from build123d import *

# Parameters (mm, degrees)
BACK_PLATE_DEPTH        = 10
BASE_PLATE_DEPTH        = 10
HOUSING_BOSS_DEPTH      = 50
MOUNTING_HOLES_REACH    = 124.984
MOUNTING_HOLES_SKETCH_R = 7.5
HOUSING_SLOT_PROFILE_W  = 28.353660078
HOUSING_SLOT_PROFILE_H  = 63.245553204
HOUSING_SLOT_CUT_DEPTH  = 20


with BuildPart() as part:
    # Back Plate Profile → Back Plate (new body)
    with BuildSketch(Plane(origin=(0, 0, 0), x_dir=(0, 0, -1), z_dir=(1, 0, 0))):
        with BuildLine():
            Line((-50, -70), (50, -70))
            Line((50, -70), (50, -60))
            Line((50, -60), (34.077790239, 7.981491866))
            ThreePointArc((34.077790239, 7.981491866), (0, 35), (-34.077790239, 7.981491866))
            Line((-34.077790239, 7.981491866), (-50, -60))
            Line((-50, -60), (-50, -70))
        make_face()
    extrude(amount=BACK_PLATE_DEPTH)

    # Base Plate Profile → Base Plate (add)
    with BuildSketch(Plane.XZ.offset(70)):
        Polygon((10, 50), (50, 50), (60, 40), (60, -40), (50, -50), (10, -50), align=None)
    extrude(amount=-BASE_PLATE_DEPTH)

    # Housing Boss Profile → Housing Boss (add)
    with BuildSketch(Plane(origin=(10, 0, 0), x_dir=(0, 0, -1), z_dir=(1, 0, 0))):
        with BuildLine():
            Line((-5, -34.641016151), (-5, -60))
            Line((-5, -60), (5, -60))
            Line((5, -60), (5, -34.641016151))
            ThreePointArc((5, -34.641016151), (0, 35), (-5, -34.641016151))
        make_face()
    extrude(amount=HOUSING_BOSS_DEPTH)

    # Mounting Holes Sketch → Mounting Holes (cut, up to next)
    with BuildSketch(Plane(origin=(0, -60, 0), x_dir=(1, 0, 0), z_dir=(0, 1, 0)), mode=Mode.PRIVATE) as mounting_holes_sk1:
        with Locations(Location((40, 35, 0), (0, 0, 270))):
            Circle(MOUNTING_HOLES_SKETCH_R)
    mounting_holes_tool1 = extrude(mounting_holes_sk1.sketch, amount=-MOUNTING_HOLES_REACH, mode=Mode.PRIVATE) & part.part
    # Mounting Holes Sketch → Mounting Holes (cut, up to next)
    with BuildSketch(Plane(origin=(0, -60, 0), x_dir=(1, 0, 0), z_dir=(0, 1, 0)), mode=Mode.PRIVATE) as mounting_holes_sk2:
        with Locations(Location((40, -35, 0), (0, 0, 270))):
            Circle(MOUNTING_HOLES_SKETCH_R)
    mounting_holes_tool2 = extrude(mounting_holes_sk2.sketch, amount=-MOUNTING_HOLES_REACH, mode=Mode.PRIVATE) & part.part
    add(mounting_holes_tool1.solids().sort_by_distance((40, -60, -35))[0], mode=Mode.SUBTRACT)
    add(mounting_holes_tool2.solids().sort_by_distance((40, -60, 35))[0], mode=Mode.SUBTRACT)

    # Gland Bore Profile → Gland Bore (revolve, cut)
    with BuildSketch(Plane.XY, mode=Mode.PRIVATE) as gland_bore_sk:
        Polygon((0, 0), (60, 0), (60, 25), (50, 25), (50, 20), (40, 20), (0, 20), align=None)
    revolve(gland_bore_sk.sketch.rotate(Axis((0, 0, 0), (1, 0, 0)), 90), axis=Axis((0, 0, 0), (1, 0, 0)), mode=Mode.SUBTRACT)

    # Housing Slot Profile → Housing Slot Cut (cut)
    with BuildSketch(Plane(origin=(60, 0, 0), x_dir=(0, 0, -1), z_dir=(1, 0, 0))):
        with Locations((-29.176830039, 0)):
            Rectangle(HOUSING_SLOT_PROFILE_W, HOUSING_SLOT_PROFILE_H)
        with Locations((29.176830039, 0)):
            Rectangle(HOUSING_SLOT_PROFILE_W, HOUSING_SLOT_PROFILE_H)
    extrude(amount=-HOUSING_SLOT_CUT_DEPTH, mode=Mode.SUBTRACT)


solid = part.part
Model file for the job. Use its own axes, mm. A direction names the side the tool comes from. Give positions to 0.01 mm unless a question says otherwise; leave off trailing zeros. Write each loop counter-clockwise with the first axis right and the second up, starting at its lowest first coordinate (ties: lowest second). Pieces come first, ordered by that corner, then holes. Notation, with made-up numbers: M -11.75,68.5 L 3.25,68.5 A24 cw 3.25,92.5 Z; hole C 35,45 d7. An arc over 180 degrees is marked long. One line per item, written item: value. Start each with the question number.
Q1. Probe probe 1 along Y at (x, z) = (33.5, -15); probe 2 along X at (y, z) = (-65.25, 35); probe 3 along Y at (x, z) = (47.5, -39.5). List the from-to ranges inside material, lowest first. Write a range as [from, to].
Q2. 3-axis set-ups, long thin cutter, end or side, ignore diameter. For faces 1 (the flat face through (10, -41, -27)), 2 (the flat face through (10, -41, 28)), 3 (the flat face through (40, 0, -25)): which of +Z, -Z, +X, -X, +Y, -Y reach the whole face in a straight line?
Q3. Saw through at B-B, the plane y = 11. Write the cut outline in (x, z).
Q4. Drop flat-ended pins along their axis: pin 1 Ø22 at (y, z) = (-11, 23.5) entering from +X; pin 2 Ø2 at (x, y) = (19, 3) entering from -Z; pin 3 Ø13.5 at (x, z) = (37.5, 31) entering from +Y. Give the stop position or say it passes through.
Q5. Saw through at A-A, the plane z = 0. Write the cut outline in (x, y), plus the area to 3 significant figures.
Q6. Saw through at C-C, the plane y = 0. Write the cut outline in (x, z).
Q7. Two-plate mould, pull along Y, no slides. Class faces 4 (the flat face through (50, 20.3, -0.2)), 5 (the flat face through (4.93, -26.49, -42.15)), 6 (the flat face through (55, -65, 45)): +Y half, -Y half, draft (parallel to the pull), parting line (faces both ways), or undercut.
Output values:
1. probe 1: y = [-70, -60], [-31.62, -13.23], [13.23, 31.62]
1. probe 2: x = [0, 32.5], [47.5, 60]
1. probe 3: y = [-70, -60]
2. face 1: -Z, +X
2. face 2: +Z, +X
2. face 3: -Z, +X, +Y
3. outline: M 0,-33.23 L 40,-33.23 L 40,-16.7 L 0,-16.7 Z; M 0,16.7 L 40,16.7 L 40,33.23 L 0,33.23 Z
4. pin 1: stops at x = 50
4. pin 2: stops at z = -34.94
4. pin 3: stops at y = 25.24
5. outline: M 0,-70 L 60,-70 L 60,-25 L 50,-25 L 50,-20 L 0,-20 Z; M 0,20 L 50,20 L 50,25 L 60,25 L 60,35 L 0,35 Z
5. area: 3,800 mm²
6. outline: M 0,-35.95 L 10,-35.95 L 10,-35 L 40,-35 L 40,-20 L 0,-20 Z; M 0,20 L 40,20 L 40,35 L 10,35 L 10,35.95 L 0,35.95 Z
7. face 4: undercut
7. face 5: +Y half
7. face 6: draft
